from build123d import *

# Parameters (mm, degrees)
SKETCH1_R           = 30
SKETCH1_R_2         = 25
BOSS_EXTRUDE1_DEPTH = 27
CHAMFER1_SIZE       = 1.5
CUT_EXTRUDE1_START  = -46.5
SKETCH2_R           = 3
CUT_EXTRUDE1_DEPTH  = 46.5


with BuildPart() as part:
    # Sketch1 → Boss-Extrude1 (new, symmetric)
    with BuildSketch(Plane.XY):
        Circle(SKETCH1_R)
        Circle(SKETCH1_R_2, mode=Mode.SUBTRACT)
    extrude(amount=BOSS_EXTRUDE1_DEPTH, both=True)

    # Chamfer1
    chamfer1_edges = [part.edges().sort_by_distance(p)[0] for p in [
        (-30, 0, -27),
        (-30, 0, 27),
        (-25, 0, -27),
        (-25, 0, 27),
    ]]
    chamfer(chamfer1_edges, length=CHAMFER1_SIZE)

    # Sketch3 → Cut-Revolve10 (revolve, cut)
    with BuildSketch(Plane(origin=(0, 0, 0), x_dir=(0, 0, -1), z_dir=(1, 0, 0))):
        with BuildLine():
            Line((-19.5, -21.5), (-19.5, -27.5))
            ThreePointArc((-19.5, -27.5), (-22.5, -24.5), (-19.5, -21.5))
        make_face()
    revolve(axis=Axis((0, -21.5, 19.5), (0, -1, 0)), mode=Mode.SUBTRACT)

    # Sketch2 → Cut-Extrude1 (cut)
    with BuildSketch(Plane(origin=(0, 0, -27), x_dir=(-1, 0, 0), z_dir=(0, 0, -1)).offset(CUT_EXTRUDE1_START)):
        with Locations((0, -24.5)):
            Circle(SKETCH2_R)
    extrude(amount=CUT_EXTRUDE1_DEPTH, mode=Mode.SUBTRACT)


solid = part.part
Could you check a few things on this model? Use its own coordinates, in mm. Round coordinates to 2 decimals unless told otherwise and drop trailing zeros. Order: outer loops, then holes, each group sorted by start corner. A loop starts at its lowest first (then second) coordinate and runs counter-clockwise, first axis right, second up. Notation, with made-up numbers: M 53,88.25 L 87,88.25 A33 cw 87,117.25 Z; hole C 41.5,19 d8. An arc over 180 degrees is marked long. One line per item, written item: value.
(1) Imagine slicing it at A-A (y = 0). Write out the boundary of the cut face in (x, z).
Ans:
outline: M -30,-25.5 L -28.5,-27 L -26.5,-27 L -25,-25.5 L -25,25.5 L -26.5,27 L -28.5,27 L -30,25.5 Z; M 25,-25.5 L 26.5,-27 L 28.5,-27 L 30,-25.5 L 30,25.5 L 28.5,27 L 26.5,27 L 25,25.5 Z
(2) I need wall thicknesses on line 1 along Y through (x, z) = (0, 12); line 2 along X through (y, z) = (-0.5, -24.5) (3 decimals); line 3 along X through (y, z) = (16, 24.5). Which ranges of each line are inside material? Lowest first, please. Write a range as from..to.
Ans:
line 1: y = -30..-27.5, 25..30
line 2: x = -29.996..-24.995, 24.995..29.996
line 3: x = -25.38..-19.21, 19.21..25.38
(3) If we mould it in two halves opening along Y, with no side actions, what happens to faces 1 (the flat face through (19, -19, -27)), 2 (the cylindrical face through (0.1, -27.5, -3.4)), 3 (the cylindrical face through (-29.97, 1.32, 0.36)), 4 (the conical face through (1.08, 25.237, -25.761))? For each: released by +Y, released by -Y, zero draft, split by the parting line, or undercut.
Ans:
face 1: zero draft
face 2: undercut
face 3: split by the parting line
face 4: undercut
(4) Imagine slicing it at B-B (x = 0). Write out the boundary of the cut face in (y, z), and give its area (3 significant figures).
Ans:
outline: M -30,-25.5 L -28.5,-27 L -27.5,-27 L -27.5,19.5 A3 cw -25,22.46 L -25,25.5 L -26.5,27 L -28.5,27 L -30,25.5 Z; M 25,-25.5 L 26.5,-27 L 28.5,-27 L 30,-25.5 L 30,25.5 L 28.5,27 L 26.5,27 L 25,25.5 Z
area: 410 mm^2
(5) I'm going to push flat-ended pins straight in: P1, Ø2, axis at x = 21.5, z = 11, coming from the -Y side; P2, Ø4, axis at y = 6, z = -10, coming from the +X side; P3, Ø3, axis at x = -0.5, z = -17, coming from the -Y side. Where does each tip first touch, or does it pass through?
Ans:
P1: stops at y = -21.9
P2: stops at x = 29.73
P3: stops at y = -30
(6) Imagine slicing it at C-C (z = 11). Write out the boundary of the cut face in (x, y), and give its area (3 significant figures).
Ans:
outline: C 0,0 d60; hole M -2.98,-24.82 A3 ccw 2.98,-24.82 A25 ccw long Z
area: 852 mm^2
